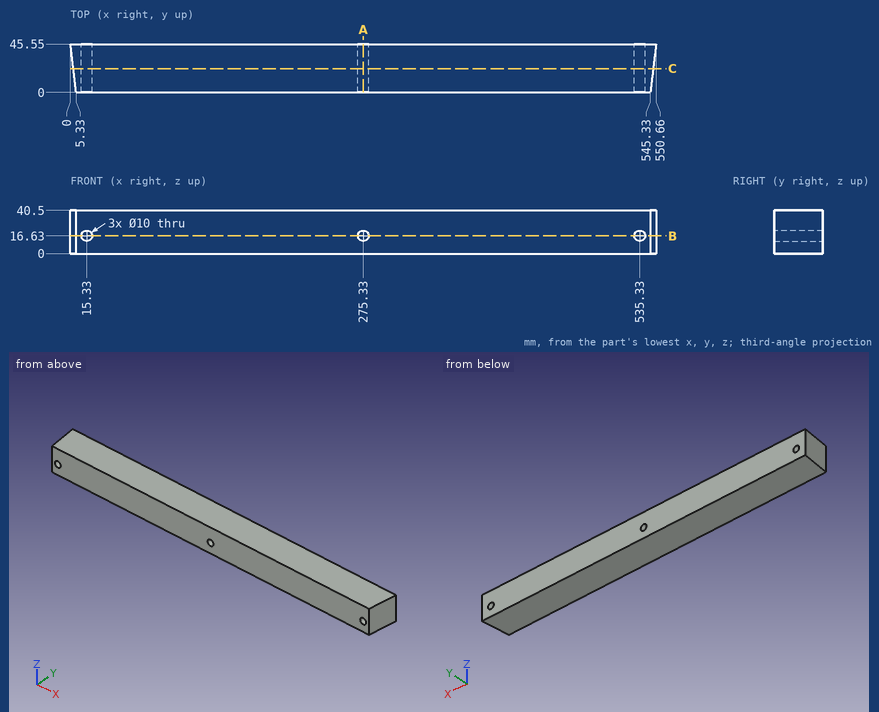
Check sheet for the drawn part. Datum: minimum x, y, z corner. Units: mm. Round coordinates to 2 decimals unless told otherwise and drop trailing zeros. Loops run counter-clockwise (first coordinate to the right, second up) from the corner with the lowest first, then second, coordinate; pieces in that order, holes last. Notation, with made-up numbers: M 70,-31 L 100,-31 A18 cw 100,-1 Z; hole C 68,26.25 d7. An arc over 180 degrees is marked long. One line per question, with ' | ' between items. Start each with the question number.
Item 1: Section check B-B (z = 16.63). Record the boundary of the cut face in (x, y), and give its area (3 significant figures).
Item 2: Gauge pin test, flat ends, axial feed: pin 1 Ø1 at (y, z) = (23, 15) entering from +X; pin 2 Ø6 at (y, z) = (29.5, 15) entering from +X; pin 3 Ø12 at (y, z) = (9, 28.5) entering from -X; pin 4 Ø9 at (x, z) = (15.33, 16.63) entering from +Y. Record the tip position at first contact, or that the pin passes through.
Item 3: Section check A-A (x = 275.33). Record the boundary of the cut face in (y, z), and give its area (3 significant figures).
Item 4: Section check C-C (y = 22.5). Record the boundary of the cut face in (x, z), and give its area (3 significant figures).
Item 5: Scan lines: probe 1 along Z at (x, y) = (275.33, 21); probe 2 along X at (y, z) = (20, 16); probe 3 along X at (y, z) = (23.5, 20). Record each from-to range of solid material in increasing order.
Worked out:
1) outline: M 0,45.55 L 5.33,0 L 10.33,0 L 10.33,45.55 Z; M 20.33,0 L 270.33,0 L 270.33,45.55 L 20.33,45.55 Z; M 280.33,0 L 530.33,0 L 530.33,45.55 L 280.33,45.55 Z; M 540.33,0 L 545.33,0 L 550.66,45.55 L 540.33,45.55 Z | area: 23,500 mm^2
2) pin 1: x = 548.08 | pin 2: x = 549.13 | pin 3: x = 3.57 | pin 4: through
3) outline: M 0,0 L 45.55,0 L 45.55,11.63 L 0,11.63 Z; M 0,21.63 L 45.55,21.63 L 45.55,40.5 L 0,40.5 Z | area: 1,390 mm^2
4) outline: M 2.7,0 L 547.96,0 L 547.96,40.5 L 2.7,40.5 Z; hole C 15.33,16.63 d10; hole C 275.33,16.63 d10; hole C 535.33,16.63 d10 | area: 21,800 mm^2
5) probe 1: 0 to 11.63, 21.63 to 40.5 | probe 2: 2.99 to 10.37, 20.29 to 270.37, 280.29 to 530.37, 540.29 to 547.67 | probe 3: 2.58 to 11.64, 19.02 to 271.64, 279.02 to 531.64, 539.02 to 548.08
